Source: CAD feature listing. Evaluate the final solid. Frame: model axes, mm. A direction names the side the tool comes from. Round coordinates to 2 decimals unless told otherwise and drop trailing zeros. Write each loop counter-clockwise with the first axis right and the second up, starting at its lowest first coordinate (ties: lowest second). Pieces come first, ordered by that corner, then holes. Notation, with made-up numbers: (-26, -20) - (10, -20) arc R16 ccw to (10, 7) - close; hole circle Ø3 at (34, -40). An arc over 180 degrees is marked (long way). Write item = value, one per line. Start each with the question number.
```python
from build123d import *

# Parameters (mm, degrees)
SKETCH_1_W      = 85
SKETCH_1_H      = 75
SKETCH_1_R      = 25.5
EXTRUDE_1_DEPTH = 8
SKETCH_2_W      = 85
SKETCH_2_H      = 10
EXTRUDE_2_DEPTH = 50


with BuildPart() as part:
    # 草图1 → 凸台-拉伸1 (new body)
    with BuildSketch(Plane.XY):
        with Locations((0, -7.5)):
            Rectangle(SKETCH_1_W, SKETCH_1_H)
        Circle(SKETCH_1_R, mode=Mode.SUBTRACT)
    extrude(amount=EXTRUDE_1_DEPTH)

    # 草图2 → 凸台-拉伸2 (add)
    with BuildSketch(Plane(origin=(0, 0, 0), x_dir=(-1, 0, 0), z_dir=(0, 0, -1))):
        with Locations((0, -40)):
            Rectangle(SKETCH_2_W, SKETCH_2_H)
    extrude(amount=EXTRUDE_2_DEPTH)


solid = part.part
```
(1) Pull-direction query (X, two-part tool) for faces 1 (the cylindrical face through (-5.5, -24.9, 3.9)), 2 (the flat face through (-42.5, -24, 1)), 3 (the flat face through (-10, -24, 0)), 4 (the flat face through (42.5, -24, 1)); classes: +X half, -X half, draft (parallel to the pull), parting line (faces both ways), or undercut.
(2) Section A-A (y = 0). Return the cut outline in (x, z), plus the area to 3 significant figures.
(3) Section C-C (x = -14). Return the cut outline in (y, z), plus the area to 3 significant figures.
(4) Section B-B (x = 0). Return the cut outline in (y, z), plus the area to 3 significant figures.
(5) Reachability of faces 5 (the flat face through (1, -45, -21)), 6 (the flat face through (1, -35, -25)) from +Z, -Z, +X, -X, +Y, -Y: full face, straight path, thin tool, end or side. Return the list, or none.
(6) Contact query for flat-ended pins moving along their axis: P1, Ø12, axis at x = 0.5, y = -22.5, coming from the -Z side; P2, Ø25, axis at x = 11.5, z = -30.5, coming from the +Y side. Output: stop coordinate, or through.
(7) Section D-D (y = 20.5). Return the cut outline in (x, z).
(8) Ray query, L1, parallel to Y at x = 0, z = 5.75; L2, parallel to Y at x = -4, z = -46; L3, parallel to Z at x = -34, y = 5.5. Return the intervals inside material, ascending. Write a range as from..to.
Solution:
q1.face_1 = undercut
q1.face_2 = -X half
q1.face_3 = draft
q1.face_4 = +X half
q2.outline = (-42.5, 0) - (-25.5, 0) - (-25.5, 8) - (-42.5, 8) - close; (25.5, 0) - (42.5, 0) - (42.5, 8) - (25.5, 8) - close
q2.area = 272 mm^2
q3.outline = (-45, -50) - (-35, -50) - (-35, 0) - (-21.31, 0) - (-21.31, 8) - (-45, 8) - close; (21.31, 0) - (30, 0) - (30, 8) - (21.31, 8) - close
q3.area = 759 mm^2
q4.outline = (-45, -50) - (-35, -50) - (-35, 0) - (-25.5, 0) - (-25.5, 8) - (-45, 8) - close; (25.5, 0) - (30, 0) - (30, 8) - (25.5, 8) - close
q4.area = 692 mm^2
q5.face_5 = +Z, -Z, +X, -X, -Y
q5.face_6 = -Z, +X, -X, +Y
q6.P1 = 0
q6.P2 = -35
q7.outline = (-42.5, 0) - (-15.17, 0) - (-15.17, 8) - (-42.5, 8) - close; (15.17, 0) - (42.5, 0) - (42.5, 8) - (15.17, 8) - close
q8.L1 = -45..-25.5, 25.5..30
q8.L2 = -45..-35
q8.L3 = 0..8
